The listing builds one solid part. Answer for the finished solid, in the listing's coordinates (mm). A direction names the side the tool comes from. Give positions to 0.01 mm unless a question says otherwise; leave off trailing zeros. Loops run counter-clockwise (first coordinate to the right, second up) from the corner with the lowest first, then second, coordinate; pieces in that order, holes last.
Item 1: Section B-B, the plane z = 0 is taken. Give the vertices of the cut face in (x, y).
Item 2: The mould has two halves that part along Z. Classify faces 3 (the face through (28.944, 38.125, -15.054)), 4 (the face through (-2.64, 5.94, 59.94)), 5 (the face through (-35, 40, 0)): pulls with the +Z half, pulls with the -Z half, needs draft (parallel to the pull), parting line crosses it, or undercut.
Item 3: Section D-D, the plane y = 13 is taken. Give the vertices of the cut face in (x, z).
Item 4: Consider line 1 along X through (y, z) = (27, 0); line 2 along X through (y, z) = (7, -1). Determine where each line is inside the solid, lowest interval first.
Item 5: Section C-C, the plane y = 5.5 is taken. Give the vertices of the cut face in (x, z), and give its area (3 significant figures).
Item 6: Each of these flat-tipped pins is pushed along its axis until it touches: pin 1 Ø12 at (y, z) = (29, -24.5) entering from -X; pin 2 Ø10 at (x, y) = (23, 19.5) entering from +Z; pin 3 Ø1.5 at (x, y) = (32, 12.5) entering from +Z. Where does it stop, or does it pass through?
Item 7: Section A-A, the plane x = 0 is taken. Give the vertices of the cut face in (y, z).
Item 8: A tool of negligible diameter and unlimited length cuts with its end or side. For faces 1 (the face through (25, 0, -25)), 2 (the face through (-41, 10, 12)), from which of +Z, -Z, +X, -X, +Y, -Y can it reach the whole face along a straight path? Write none if from no direction.
from build123d import *

# Parameters (mm, degrees)
CHAMFER1_SIZE = 2


with BuildPart() as part:
    # Sketch1 → Revolve1 (revolve)
    with BuildSketch(Plane.XY, mode=Mode.PRIVATE) as revolve1_sk:
        Polygon((-32.5, 0), (-32.5, 40), (-42.5, 40), (-42.5, 10), (-60, 10), (-60, 0), align=None)
    revolve(revolve1_sk.sketch.rotate(Axis((0, 0, 0), (0, 1, 0)), 270), axis=Axis((0, 0, 0), (0, 1, 0)))

    # Chamfer1
    chamfer1_edges = [part.edges().sort_by_distance(p)[0] for p in [
        (0, 0, 60),
        (0, 40, 32.5),
        (0, 0, 32.5),
    ]]
    chamfer(chamfer1_edges, length=CHAMFER1_SIZE)


solid = part.part
Worked answers:
1. outline: (-60, 2) - (-58, 0) - (-34.5, 0) - (-32.5, 2) - (-32.5, 38) - (-34.5, 40) - (-42.5, 40) - (-42.5, 10) - (-60, 10) - close; (32.5, 2) - (34.5, 0) - (58, 0) - (60, 2) - (60, 10) - (42.5, 10) - (42.5, 40) - (34.5, 40) - (32.5, 38) - close
2. face 3: undercut
2. face 4: parting line crosses it
2. face 5: needs draft
3. outline: circle Ø85 at (0, 0); hole circle Ø65 at (0, 0)
4. line 1: x = -42.5 to -32.5, 32.5 to 42.5
4. line 2: x = -59.99 to -32.48, 32.48 to 59.99
5. outline: circle Ø120 at (0, 0); hole circle Ø65 at (0, 0)
5. area: 7,990 mm2
6. pin 1: stops at x = -38.26
6. pin 2: stops at z = 38.5
6. pin 3: stops at z = 28.8
7. outline: (0, -58) - (2, -60) - (10, -60) - (10, -42.5) - (40, -42.5) - (40, -34.5) - (38, -32.5) - (2, -32.5) - (0, -34.5) - close; (0, 34.5) - (2, 32.5) - (38, 32.5) - (40, 34.5) - (40, 42.5) - (10, 42.5) - (10, 60) - (2, 60) - (0, 58) - close
8. face 1: +Z, -Z, +X, -X, -Y
8. face 2: +Y
